from build123d import *

# Parameters (mm, degrees)
SKETCH1_W                                           = 64.8
SKETCH1_H                                           = 20
BOSS_EXTRUDE1_DEPTH                                 = 23
SKETCH2_R                                           = 1.5
CUT_EXTRUDE1_DEPTH                                  = 20
CBORE_FOR_M8_HEX_SOCKET_HEAD_CAP_SCREW1_D           = 9
CBORE_FOR_M8_HEX_SOCKET_HEAD_CAP_SCREW1_DEPTH       = 41.94
CBORE_FOR_M8_HEX_SOCKET_HEAD_CAP_SCREW1_CBORE_D     = 15
CBORE_FOR_M8_HEX_SOCKET_HEAD_CAP_SCREW1_CBORE_DEPTH = 8.6
CBORE_FOR_M8_HEX_SOCKET_HEAD_CAP_SCREW1_TIP         = 2.703872786
CBORE_FOR_M3_HEX_SOCKET_HEAD_CAP_SCREW1_D           = 3.4
CBORE_FOR_M3_HEX_SOCKET_HEAD_CAP_SCREW1_DEPTH       = 41.94
CBORE_FOR_M3_HEX_SOCKET_HEAD_CAP_SCREW1_CBORE_D     = 6.5
CBORE_FOR_M3_HEX_SOCKET_HEAD_CAP_SCREW1_CBORE_DEPTH = 3.4
CBORE_FOR_M3_HEX_SOCKET_HEAD_CAP_SCREW1_TIP         = 1.021463052


with BuildPart() as part:
    # Sketch1 → Boss-Extrude1 (new body)
    with BuildSketch(Plane(origin=(0, 0, 0), x_dir=(1, 0, 0), z_dir=(0, 1, 0))):
        Rectangle(SKETCH1_W, SKETCH1_H)
    extrude(amount=BOSS_EXTRUDE1_DEPTH)

    # Sketch2 → Cut-Extrude1 (cut)
    with BuildSketch(Plane(origin=(0, 0, 0), x_dir=(1, 0, 0), z_dir=(0, 1, 0))):
        with Locations(Location((18.9, -6, 0), (0, 0, 270))):
            Circle(SKETCH2_R)
    extrude(amount=CUT_EXTRUDE1_DEPTH, mode=Mode.SUBTRACT)

    # CBORE for M8 Hex Socket Head Cap Screw1
    with Locations(Plane(origin=(-22.4, 11.5, -10), x_dir=(-1, 0, 0), z_dir=(0, 0, -1))):
        with Locations((0, 0), (-29.8, 0)):
            CounterBoreHole(CBORE_FOR_M8_HEX_SOCKET_HEAD_CAP_SCREW1_D / 2, CBORE_FOR_M8_HEX_SOCKET_HEAD_CAP_SCREW1_CBORE_D / 2, CBORE_FOR_M8_HEX_SOCKET_HEAD_CAP_SCREW1_CBORE_DEPTH, depth=CBORE_FOR_M8_HEX_SOCKET_HEAD_CAP_SCREW1_DEPTH)
            with Locations((0, 0, -(CBORE_FOR_M8_HEX_SOCKET_HEAD_CAP_SCREW1_DEPTH + CBORE_FOR_M8_HEX_SOCKET_HEAD_CAP_SCREW1_TIP / 2))):  # 118° drill point
                Cone(0, CBORE_FOR_M8_HEX_SOCKET_HEAD_CAP_SCREW1_D / 2, CBORE_FOR_M8_HEX_SOCKET_HEAD_CAP_SCREW1_TIP, mode=Mode.SUBTRACT)

    # CBORE for M3 Hex Socket Head Cap Screw1
    with Locations(Plane(origin=(-7.5, 11.5, -10), x_dir=(-1, 0, 0), z_dir=(0, 0, -1))):
        with Locations((0, 0)):
            CounterBoreHole(CBORE_FOR_M3_HEX_SOCKET_HEAD_CAP_SCREW1_D / 2, CBORE_FOR_M3_HEX_SOCKET_HEAD_CAP_SCREW1_CBORE_D / 2, CBORE_FOR_M3_HEX_SOCKET_HEAD_CAP_SCREW1_CBORE_DEPTH, depth=CBORE_FOR_M3_HEX_SOCKET_HEAD_CAP_SCREW1_DEPTH)
            with Locations((0, 0, -(CBORE_FOR_M3_HEX_SOCKET_HEAD_CAP_SCREW1_DEPTH + CBORE_FOR_M3_HEX_SOCKET_HEAD_CAP_SCREW1_TIP / 2))):  # 118° drill point
                Cone(0, CBORE_FOR_M3_HEX_SOCKET_HEAD_CAP_SCREW1_D / 2, CBORE_FOR_M3_HEX_SOCKET_HEAD_CAP_SCREW1_TIP, mode=Mode.SUBTRACT)


solid = part.part
Build history of the part. All positions in model axes, mm. A direction names the side the tool comes from. Coordinates: 2 decimals unless noted, no trailing zeros. Order: outer loops, then holes, each group sorted by start corner. A loop starts at its lowest first (then second) coordinate and runs counter-clockwise, first axis right, second up. Notation, with made-up numbers: (31.25, 54) - (45.25, 54) arc R12 ccw to (45.25, 69) - close; hole circle Ø1 at (-3, -23.75). An arc over 180 degrees is marked (long way). Write item = value, one per line. Start each with the question number.
1) 3-axis set-ups, long thin cutter, end or side, ignore diameter. For faces 1 (the face through (-25.861, 4.846, -5.76)), 2 (the face through (19, 20, 6)), 3 (the face through (0, 11, 10)): which of +Z, -Z, +X, -X, +Y, -Y reach the whole face in a straight line?
2) Saw through at D-D on x = 7.4. Write the cut outline in (y, z), then the cut area to 3 significant figures.
3) Flat gauge pins, fed straight in: pin 1 Ø12 at (x, y) = (-22.4, 11.5) entering from -Z; pin 2 Ø5.5 at (x, y) = (-22.4, 11.5) entering from -Z; pin 3 Ø3 at (x, y) = (-7, 11) entering from -Z. Where does each tip first touch, or does it go through?
4) Saw through at A-A on y = 11.5. Count the separate pieces of the cut face and the enclosed holes in it, then the cut area to 3 significant figures.
5) Wall check: line 1 along Y through (x, z) = (7.4, 3.75); line 2 along X through (y, z) = (6, -8.5); line 3 along Y through (x, z) = (-7.5, 1.75). Give the ranges that are in metal, low to high. Write a range as from..to.
6) Two-plate mould, pull along Z, no slides. Class faces 4 (the face through (-0.5, 11.3, -10)), 5 (the face through (19.91, 9.86, 4.89)), 6 (the face through (-7.721, 13.186, 1.816)): pulls with the +Z half, pulls with the -Z half, needs draft (parallel to the pull), parting line crosses it, or undercut.
7) Saw through at C-C on z = 6. Write the cut outline in (x, y), then the cut area to 3 significant figures.
8) Saw through at B-B on x = -7.5. Write the cut outline in (y, z), then the cut area to 3 significant figures.
From the geometry:
q1.face_1 = -Z
q1.face_2 = -Y
q1.face_3 = +Z, +X, -X, +Y, -Y
q2.outline = (0, -10) - (4, -10) - (4, -1.4) - (7, -1.4) - (7, 10) - (0, 10) - close; (16, -1.4) - (19, -1.4) - (19, -10) - (23, -10) - (23, 10) - (16, 10) - close
q2.area = 228 mm^2
q3.pin_1 = -1.4
q3.pin_2 = through
q3.pin_3 = -6.6
q4.separate_pieces = 4
q4.enclosed_holes = 1
q4.area = 747 mm^2
q5.line_1 = 0..7, 16..23
q5.line_2 = -32.4..-27.5, -17.3..2.3, 12.5..32.4
q5.line_3 = 0..9.8, 13.2..23
q6.face_4 = pulls with the -Z half
q6.face_5 = undercut
q6.face_6 = needs draft
q7.outline = (-32.4, 0) - (17.4, 0) - (17.4, 20) - (20.4, 20) - (20.4, 0) - (32.4, 0) - (32.4, 23) - (-32.4, 23) - close; hole circle Ø9 at (-22.4, 11.5); hole circle Ø3.4 at (-7.5, 11.5); hole circle Ø9 at (7.4, 11.5)
q7.area = 1,290 mm^2
q8.outline = (0, -10) - (8.25, -10) - (8.25, -6.6) - (9.8, -6.6) - (9.8, 10) - (0, 10) - close; (13.2, -6.6) - (14.75, -6.6) - (14.75, -10) - (23, -10) - (23, 10) - (13.2, 10) - close
q8.area = 381 mm^2
